```python
from build123d import *

# Parameters (mm, degrees)
SKETCH1_W                                           = 700
SKETCH1_H                                           = 18
BOSS_EXTRUDE1_DEPTH                                 = 16.5
SKETCH4_W                                           = 700
SKETCH4_H                                           = 15
CUT_EXTRUDE1_DEPTH                                  = 3
M4_TAPPED_HOLE1_D                                   = 3.3
M4_TAPPED_HOLE1_DEPTH                               = 15.5
M4_TAPPED_HOLE1_TIP                                 = 0.991420021
CBORE_FOR_M5_HEX_SOCKET_HEAD_CAP_SCREW1_D           = 5.5
CBORE_FOR_M5_HEX_SOCKET_HEAD_CAP_SCREW1_CBORE_D     = 10
CBORE_FOR_M5_HEX_SOCKET_HEAD_CAP_SCREW1_CBORE_DEPTH = 18
SIZE_MM_DOWEL_HOLE_1_D                              = 8
SIZE_MM_DOWEL_HOLE_1_DEPTH                          = 11
SIZE_MM_DOWEL_HOLE_1_TIP                            = 2.403442476
CHAMFER1_SIZE                                       = 1


with BuildPart() as part:
    # Sketch1 → Boss-Extrude1 (new, symmetric)
    with BuildSketch(Plane.XY):
        Rectangle(SKETCH1_W, SKETCH1_H)
    extrude(amount=BOSS_EXTRUDE1_DEPTH, both=True)

    # Sketch4 → Cut-Extrude1 (cut)
    with BuildSketch(Plane.XY.offset(16.5)):
        with Locations((0, 1.5)):
            Rectangle(SKETCH4_W, SKETCH4_H)
    extrude(amount=-CUT_EXTRUDE1_DEPTH, mode=Mode.SUBTRACT)

    # M4 Tapped Hole1
    with Locations(Plane.XY.offset(13.5)):
        with Locations((330, 1.5), (270, 1.5), (210, 1.5), (150, 1.5), (90, 1.5), (30, 1.5), (-30, 1.5), (-90, 1.5), (-150, 1.5), (-330, 1.5), (-210, 1.5), (-270, 1.5)):
            Hole(M4_TAPPED_HOLE1_D / 2, depth=M4_TAPPED_HOLE1_DEPTH)
            with Locations((0, 0, -(M4_TAPPED_HOLE1_DEPTH + M4_TAPPED_HOLE1_TIP / 2))):  # 118° drill point
                Cone(0, M4_TAPPED_HOLE1_D / 2, M4_TAPPED_HOLE1_TIP, mode=Mode.SUBTRACT)

    # CBORE for M5 Hex Socket Head Cap Screw1 (through all)
    with Locations(Plane.XY.offset(16.5)):
        with Locations((-342, 0), (-240, 0), (-120, 0), (0, 0), (120, 0), (240, 0), (342, 0)):
            CounterBoreHole(CBORE_FOR_M5_HEX_SOCKET_HEAD_CAP_SCREW1_D / 2, CBORE_FOR_M5_HEX_SOCKET_HEAD_CAP_SCREW1_CBORE_D / 2, CBORE_FOR_M5_HEX_SOCKET_HEAD_CAP_SCREW1_CBORE_DEPTH)

    # Size mm dowel hole 1
    with Locations(Plane(origin=(0, 0, -16.5), x_dir=(-1, 0, 0), z_dir=(0, 0, -1))):
        with Locations((-300, 0), (300, 0)):
            Hole(SIZE_MM_DOWEL_HOLE_1_D / 2, depth=SIZE_MM_DOWEL_HOLE_1_DEPTH)
            with Locations((0, 0, -(SIZE_MM_DOWEL_HOLE_1_DEPTH + SIZE_MM_DOWEL_HOLE_1_TIP / 2))):  # 118° drill point
                Cone(0, SIZE_MM_DOWEL_HOLE_1_D / 2, SIZE_MM_DOWEL_HOLE_1_TIP, mode=Mode.SUBTRACT)

    # Chamfer1
    chamfer1_edges = [part.edges().sort_by_distance(p)[0] for p in [
        (-350, 9, -1.5),
        (350, 9, -1.5),
        (350, -9, 0),
        (-350, -9, 0),
    ]]
    chamfer(chamfer1_edges, length=CHAMFER1_SIZE)


solid = part.part
```
The listing builds one solid part. Answer for the finished solid, in the listing's coordinates (mm). A direction names the side the tool comes from. Give positions to 0.01 mm unless a question says otherwise; leave off trailing zeros. Order: outer loops, then holes, each group sorted by start corner. A loop starts at its lowest first (then second) coordinate and runs counter-clockwise, first axis right, second up. Notation, with made-up numbers: M 84,-38.75 L 100,-38.75 A25 ccw 100,-24.75 Z; hole C 33.5,84 d11. An arc over 180 degrees is marked long. Put each result on its own line as item: value. Start each with the question number.
Item 1: Find the intervals of material crossed by line 1 along Y through (x, z) = (120, 7.75); line 2 along Y through (x, z) = (-330, 10); line 3 along Z through (x, y) = (228, 7), in increasing order.
Item 2: Which of the six approach directions +Z, -Z, +X, -X, +Y, -Y give full straight-line access (tool end or side, diameter ignored) to faces 1 (the face through (350, 0, 0)), 2 (the face through (-5, 2, 13.5))?
Item 3: Flat-ended cylindrical pins translate along their axes: P1, Ø8, axis at x = -217, y = 2, coming from the +Z side; P2, Ø3, axis at x = 30, y = 1.5, coming from the +Z side; P3, Ø6, axis at x = 120, y = 0, coming from the +Z side. Find the tip coordinate at first contact, or state that the pin passes through.
Item 4: The part is cut by section A-A, the plane x = 255. Determine the outline of the cut face in (y, z).
Answer key:
1. line 1: y = -9 to -5, 5 to 9
1. line 2: y = -9 to -0.15, 3.15 to 9
1. line 3: z = -16.5 to 13.5
2. face 1: +Z, -Z, +X, +Y, -Y
2. face 2: +Z, +X, -X, +Y
3. P1: stops at z = 13.5
3. P2: stops at z = -2.09
3. P3: stops at z = -1.5
4. outline: M -9,-16.5 L 9,-16.5 L 9,13.5 L -6,13.5 L -6,16.5 L -9,16.5 Z
